Study the drawing (mm; zero at the part's minimum x, y, z) and answer. Coordinates: 2 decimals unless noted, no trailing zeros. Order: outer loops, then holes, each group sorted by start corner. A loop starts at its lowest first (then second) coordinate and runs counter-clockwise, first axis right, second up.
1. The part is cut by section A-A, the plane x = 9. Count the separate pieces of the cut face and the enclosed holes in it, then the cut area to 3 significant figures.
2. Flat-ended cylindrical pins translate along their axes: pin 1 Ø2 at (x, y) = (23.5, 6.5) entering from -Z; pin 2 Ø3 at (x, y) = (3.5, 6) entering from +Z. Find the tip coordinate at first contact, or state that the pin passes through.
3. The part is cut by section B-B, the plane y = 15. Give the vertices of the cut face in (x, z).
4. Find the intervals of material crossed by probe 1 along Y at (x, z) = (4, 0.6); probe 2 along Y at (x, z) = (2.5, 0.6); probe 3 along X at (y, z) = (18.75, 1.45), in increasing order.
5. The part is cut by section D-D, the plane y = 3. Give the vertices of the cut face in (x, z), then the cut area to 3 significant figures.
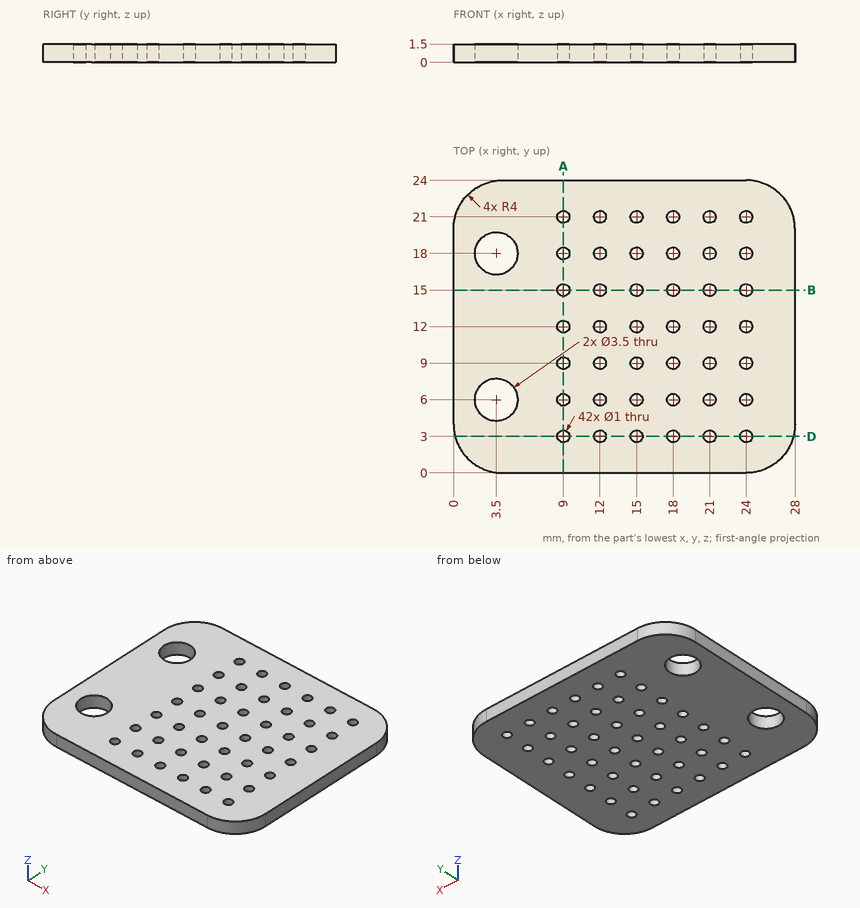
Geometry says:
1. separate pieces: 8
1. enclosed holes: 0
1. area: 25.5 mm2
2. pin 1: stops at z = 0
2. pin 2: passes through
3. outline: (0, 0) - (8.5, 0) - (8.5, 1.5) - (0, 1.5) - close; (9.5, 0) - (11.5, 0) - (11.5, 1.5) - (9.5, 1.5) - close; (12.5, 0) - (14.5, 0) - (14.5, 1.5) - (12.5, 1.5) - close; (15.5, 0) - (17.5, 0) - (17.5, 1.5) - (15.5, 1.5) - close; (18.5, 0) - (20.5, 0) - (20.5, 1.5) - (18.5, 1.5) - close; (21.5, 0) - (23.5, 0) - (23.5, 1.5) - (21.5, 1.5) - close; (24.5, 0) - (28, 0) - (28, 1.5) - (24.5, 1.5) - close
4. probe 1: y = 0 to 4.32, 7.68 to 16.32, 19.68 to 24
4. probe 2: y = 0.29 to 4.56, 7.44 to 16.56, 19.44 to 23.71
4. probe 3: x = 0 to 1.92, 5.08 to 28
5. outline: (0.13, 0) - (8.5, 0) - (8.5, 1.5) - (0.13, 1.5) - close; (9.5, 0) - (11.5, 0) - (11.5, 1.5) - (9.5, 1.5) - close; (12.5, 0) - (14.5, 0) - (14.5, 1.5) - (12.5, 1.5) - close; (15.5, 0) - (17.5, 0) - (17.5, 1.5) - (15.5, 1.5) - close; (18.5, 0) - (20.5, 0) - (20.5, 1.5) - (18.5, 1.5) - close; (21.5, 0) - (23.5, 0) - (23.5, 1.5) - (21.5, 1.5) - close; (24.5, 0) - (27.87, 0) - (27.87, 1.5) - (24.5, 1.5) - close
5. area: 32.6 mm2
